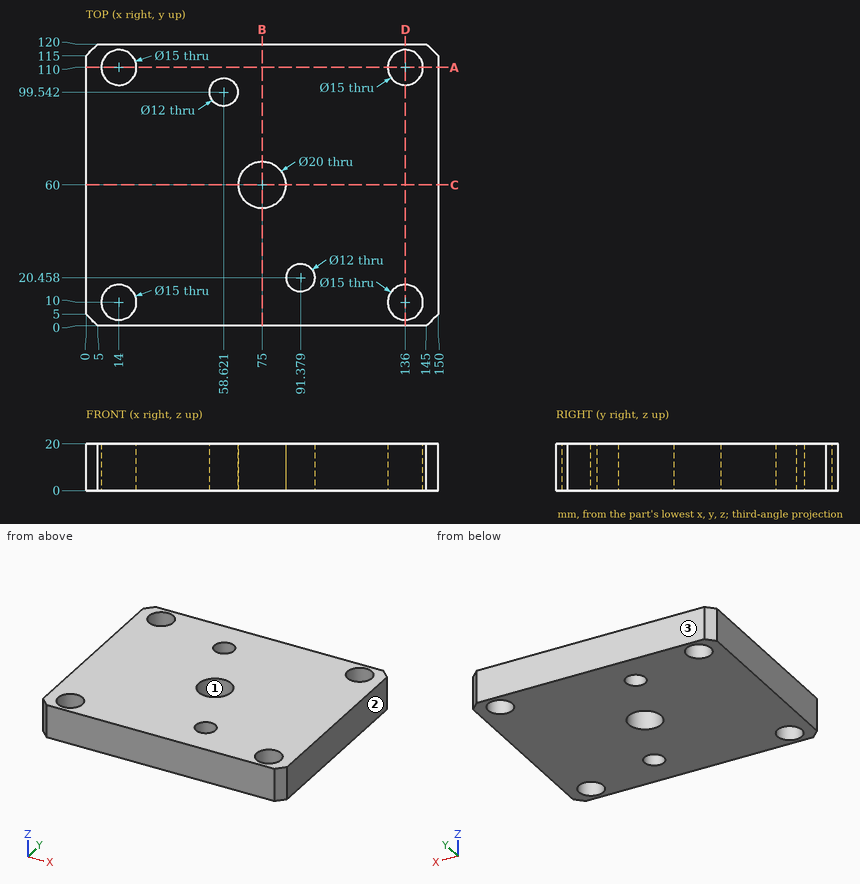
Job drawing, mm, ordinate dimensions from the low corner. One solid piece. Give positions to 0.01 mm unless a question says otherwise; leave off trailing zeros. Loops run counter-clockwise (first coordinate to the right, second up) from the corner with the lowest first, then second, coordinate; pieces in that order, holes last. Notation, with made-up numbers: (19.25, 27.25) - (55.25, 27.25) arc R12 cw to (55.25, 45.25) - close; hole circle Ø11 at (88.25, 59). An arc over 180 degrees is marked (long way). Use one line per item in the form item = value.
(1) Drop a flat-ended pin along its axis: P1, Ø12, axis at x = 136, y = 10, coming from the -Z side. Give the stop position or say it passes through.
Determined:
P1 = through
(2) Cut at C-C (y = 60). Give the cut face in (x, z).
Determined:
outline = (0, 0) - (65, 0) - (65, 20) - (0, 20) - close; (85, 0) - (150, 0) - (150, 20) - (85, 20) - close
(3) Cut at A-A (y = 110). Give the cut face in (x, z).
Determined:
outline = (0, 0) - (6.5, 0) - (6.5, 20) - (0, 20) - close; (21.5, 0) - (128.5, 0) - (128.5, 20) - (21.5, 20) - close; (143.5, 0) - (150, 0) - (150, 20) - (143.5, 20) - close
(4) Drill centre lines: L1, parallel to X at y = 10.5, z = 5.25; L2, parallel to Y at x = 136, z = 7.5; L3, parallel to X at y = 111, z = 4.25. Where is each one in solid material? Low to high.
Determined:
L1 = 0 to 6.52, 21.48 to 128.52, 143.48 to 150
L2 = 0 to 2.5, 17.5 to 102.5, 117.5 to 120
L3 = 0 to 6.57, 21.43 to 128.57, 143.43 to 150
(5) Cut at D-D (x = 136). Give the cut face in (y, z).
Determined:
outline = (0, 0) - (2.5, 0) - (2.5, 20) - (0, 20) - close; (17.5, 0) - (102.5, 0) - (102.5, 20) - (17.5, 20) - close; (117.5, 0) - (120, 0) - (120, 20) - (117.5, 20) - close
(6) Pull direction Y, two halves, no side cores. Call the marked faces 1, 2 and 3: pulls with the +Y half, pulls with the -Y half, needs draft (parallel to the pull), parting line crosses it, or undercut.
Determined:
face_1 = undercut
face_2 = needs draft
face_3 = pulls with the +Y half
(7) Cut at B-B (x = 75). Give the cut face in (y, z), then the cut area to 3 significant figures.
Determined:
outline = (0, 0) - (50, 0) - (50, 20) - (0, 20) - close; (70, 0) - (120, 0) - (120, 20) - (70, 20) - close
area = 2,000 mm^2
